Geometry: final body of the model. Coordinates: model frame, mm. Face numbers are marked on the shaded views. A direction names the side the tool comes from. Give positions to 0.01 mm unless a question says otherwise; leave off trailing zeros. Loops run counter-clockwise (first coordinate to the right, second up) from the corner with the lowest first, then second, coordinate; pieces in that order, holes last. Notation, with made-up numbers: (25, -4.5) -> (34, -4.5) arc R29 ccw to (34, 24.5) -> close; hole circle Ø4 at (18, 84.5). An arc over 180 degrees is marked (long way). Answer in a Markdown table with one row per item. Add a question column.
from build123d import *

# Parameters (mm, degrees)
SKETCH_1_W                     = 110
SKETCH_1_H                     = 110
EXTRUDE_1_DEPTH                = 14
SKETCH_2_R                     = 40
SKETCH_2_R_2                   = 38
EXTRUDE_2_DEPTH                = 2
SKETCH_3_R                     = 38
CUT_EXTRUDE_1_DEPTH            = 80.031639234
SKETCH_4_R                     = 42.5
CUT_EXTRUDE_2_DEPTH            = 3.1
HOLE_WIZARD_M8_1_D             = 6.8
HOLE_WIZARD_M8_1_2_D           = 9
HOLE_WIZARD_M8_1_2_CBORE_D     = 15
HOLE_WIZARD_M8_1_2_CBORE_DEPTH = 8.6
CHAMFER_1_SIZE                 = 5
CHAMFER_2_SIZE                 = 0.5


with BuildPart() as part:
    # 草图1 → 凸台-拉伸1 (new body)
    with BuildSketch(Plane.XY):
        Rectangle(SKETCH_1_W, SKETCH_1_H)
    extrude(amount=EXTRUDE_1_DEPTH)

    # 草图2 → 凸台-拉伸2 (add)
    with BuildSketch(Plane.XY.offset(14)):
        with Locations(Location((0, 0, 0), (0, 0, 180))):
            Circle(SKETCH_2_R)
        Circle(SKETCH_2_R_2, mode=Mode.SUBTRACT)
    extrude(amount=EXTRUDE_2_DEPTH)

    # 草图3 → 切除-拉伸1 (cut, through all)
    with BuildSketch(Plane.XY.offset(14)):
        Circle(SKETCH_3_R)
    extrude(amount=-CUT_EXTRUDE_1_DEPTH, mode=Mode.SUBTRACT)

    # 草图4 → 切除-拉伸2 (cut)
    with BuildSketch(Plane(origin=(0, 0, 0), x_dir=(-1, 0, 0), z_dir=(0, 0, -1))):
        Circle(SKETCH_4_R)
    extrude(amount=-CUT_EXTRUDE_2_DEPTH, mode=Mode.SUBTRACT)

    # Hole Wizard M8 _1 (through all)
    with Locations(Plane(origin=(0, 0, 0), x_dir=(-1, 0, 0), z_dir=(0, 0, -1))):
        with Locations((-44.5, 44.5), (0, 0), (44.5, 44.5), (-44.5, -44.5), (44.5, -44.5)):
            Hole(HOLE_WIZARD_M8_1_D / 2)

    # Hole Wizard M8 _1 2 (through all)
    with Locations(Plane(origin=(0, 0, 0), x_dir=(-1, 0, 0), z_dir=(0, 0, -1))):
        with Locations((36, -36), (36, 36), (-36, -36), (-36, 36)):
            CounterBoreHole(HOLE_WIZARD_M8_1_2_D / 2, HOLE_WIZARD_M8_1_2_CBORE_D / 2, HOLE_WIZARD_M8_1_2_CBORE_DEPTH)

    # 倒角1
    chamfer_1_edges = [part.edges().sort_by_distance(p)[0] for p in [
        (55, -55, 7),
        (-55, -55, 7),
        (-55, 55, 7),
        (55, 55, 7),
    ]]
    chamfer(chamfer_1_edges, length=CHAMFER_1_SIZE)

    # 倒角2
    chamfer_2_edges = [part.edges().sort_by_distance(p)[0] for p in [
        (40, 0, 16),
        (42.5, 0, 0),
    ]]
    chamfer(chamfer_2_edges, length=CHAMFER_2_SIZE)


solid = part.part
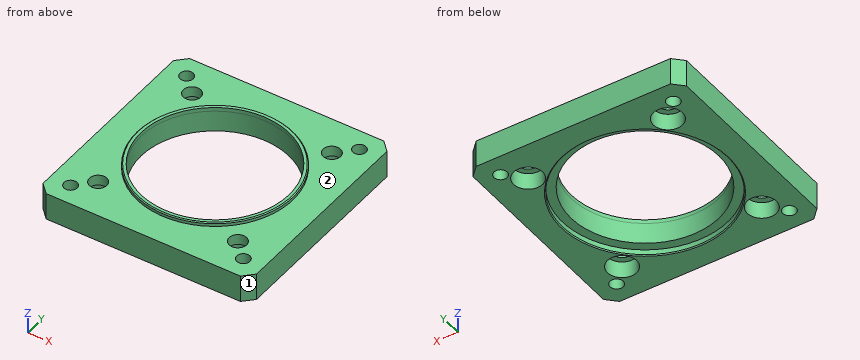
(1) Reachability of the marked faces 1 and 2 from +Z, -Z, +X, -X, +Y, -Y: full face, straight path, thin tool, end or side. Return the list, or none.
(2) Cut plane A-A on z = 7. State how many separate pieces and enclosed holes the cut face has, then the cut area to 3 significant figures.
(3) Cut plane B-B on x = 0. Return the cut outline in (y, z), then the cut area to 3 significant figures.
(4) Pin query (flat end, axial travel): pin 1 Ø14.5 at (x, y) = (36, 36) entering from -Z; pin 2 Ø14.5 at (x, y) = (36, -36) entering from +Z. Return the tip coordinate at first contact, or that it passes through.
(5) Material intervals for line 1 along Y through (x, z) = (44.5, 8.5); line 2 along Y through (x, z) = (0, 1.6); line 3 along Y through (x, z) = (0, 14.6), sorted ascending. Write a range as from..to.
Answer list:
| question | item | result |
|---|---|---|
| 1 | face 1 | +Z, -Z, +X, -Y |
| 1 | face 2 | +Z |
| 2 | separate pieces | 1 |
| 2 | enclosed holes | 9 |
| 2 | area | 6,660 mm² |
| 3 | outline | (-55, 0) -> (-43, 0) -> (-42.5, 0.5) -> (-42.5, 3.1) -> (-38, 3.1) -> (-38, 16) -> (-39.5, 16) -> (-40, 15.5) -> (-40, 14) -> (-55, 14) -> close; (38, 3.1) -> (42.5, 3.1) -> (42.5, 0.5) -> (43, 0) -> (55, 0) -> (55, 14) -> (40, 14) -> (40, 15.5) -> (39.5, 16) -> (38, 16) -> close |
| 3 | area | 456 mm² |
| 4 | pin 1 | stops at z = 8.6 |
| 4 | pin 2 | stops at z = 14 |
| 5 | line 1 | y = -55..-47.9, -41.1..41.1, 47.9..55 |
| 5 | line 2 | y = -55..-42.5, 42.5..55 |
| 5 | line 3 | y = -40..-38, 38..40 |
